Here's how the part is built. I have some questions about the finished solid (model axes, mm). Face numbers are marked on the shaded views. A direction names the side the tool comes from. Coordinates: 2 decimals unless noted, no trailing zeros. Write each loop counter-clockwise with the first axis right and the second up, starting at its lowest first coordinate (ties: lowest second). Pieces come first, ordered by that corner, then holes. Notation, with made-up numbers: (59, 75.25) -> (78, 75.25) arc R25 cw to (78, 88.25) -> close; hole circle Ø4 at (63.5, 36.25). An arc over 180 degrees is marked (long way). Put each result on its own line as item: value. Start each with the question number.
Item 1: I need wall thicknesses on line 1 (X direction, y = 24.5, z = 0.3); line 2 (Y direction, x = 17.5, z = 1.35); line 3 (X direction, y = 32.5, z = 2.7). Which ranges of each line are inside material? Lowest first, please. Write a range as [from, to].
Item 2: I want a section at B-B, the plane y = 29.5. List the corners of the cut face in (x, z) for me.
Item 3: If we mould it in two halves opening along Y, with no side actions, what happens to the marked faces 3, 4 and 5? For each: released by +Y, released by -Y, zero draft, split by the parting line, or undercut.
Item 4: On a 3-axis mill with a long thin cutter (end or side, diameter ignored), from which of +Z, -Z, +X, -X, +Y, -Y can I reach the whole of each face in a straight line? I mean the marked faces 1 and 2. Say none if no direction works.
Item 5: I want a section at C-C, the plane z = 2.15. List the corners of the cut face in (x, y) for me, then the cut area to 3 significant figures.
Item 6: I want a section at A-A, the plane x = 17.5. List the corners of the cut face in (y, z) for me.
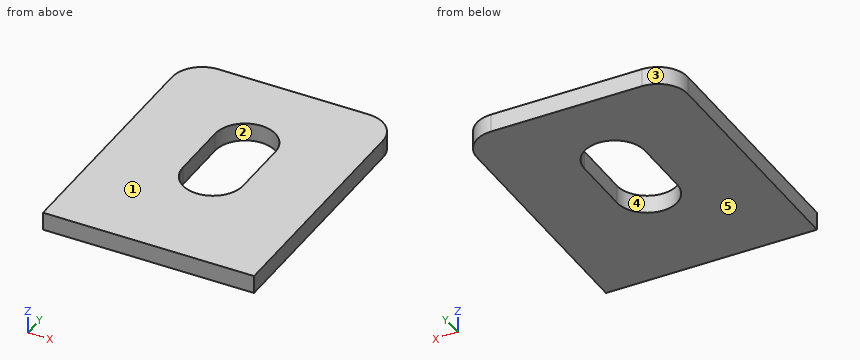
from build123d import *

# Parameters (mm, degrees)
BOSS_EXTRUDE1_DEPTH = 3


with BuildPart() as part:
    # Sketch1 → Boss-Extrude1 (new body)
    with BuildSketch(Plane.XY):
        with BuildLine():
            Line((0, 0), (35, 0))
            Line((35, 0), (35, 40))
            ThreePointArc((35, 40), (33.535533906, 43.535533906), (30, 45))
            Line((30, 45), (5, 45))
            ThreePointArc((5, 45), (1.464466094, 43.535533906), (0, 40))
            Line((0, 40), (0, 0))
        make_face()
        with BuildLine():
            Line((12.5, 30), (12.5, 20))
            ThreePointArc((12.5, 20), (17.5, 15), (22.5, 20))
            Line((22.5, 20), (22.5, 30))
            ThreePointArc((22.5, 30), (17.5, 35), (12.5, 30))
        make_face(mode=Mode.SUBTRACT)
    extrude(amount=BOSS_EXTRUDE1_DEPTH)


solid = part.part
Calculated:
1. line 1: x = [0, 12.5], [22.5, 35]
1. line 2: y = [0, 15], [35, 45]
1. line 3: x = [0, 13.17], [21.83, 35]
2. outline: (0, 0) -> (12.5, 0) -> (12.5, 3) -> (0, 3) -> close; (22.5, 0) -> (35, 0) -> (35, 3) -> (22.5, 3) -> close
3. face 3: released by +Y
3. face 4: undercut
3. face 5: zero draft
4. face 1: +Z, +X, -X, +Y, -Y
4. face 2: +Z, -Z
5. outline: (0, 0) -> (35, 0) -> (35, 40) arc R5 ccw to (30, 45) -> (5, 45) arc R5 ccw to (0, 40) -> close; hole (12.5, 20) arc R5 ccw to (22.5, 20) -> (22.5, 30) arc R5 ccw to (12.5, 30) -> close
5. area: 1,390 mm2
6. outline: (0, 0) -> (15, 0) -> (15, 3) -> (0, 3) -> close; (35, 0) -> (45, 0) -> (45, 3) -> (35, 3) -> close
